Source: CAD feature listing. Evaluate the final solid. Frame: model axes, mm. A direction names the side the tool comes from. Give positions to 0.01 mm unless a question says otherwise; leave off trailing zeros. Order: outer loops, then holes, each group sorted by start corner. A loop starts at its lowest first (then second) coordinate and runs counter-clockwise, first axis right, second up.
```python
from build123d import *

# Parameters (mm, degrees)
EXTRUDE_1_DEPTH = 180


with BuildPart() as part:
    # 草图1 → 凸台-拉伸1 (new body)
    with BuildSketch(Plane.XY):
        Polygon((0, 0), (110, 0), (110, -30), (102, -30), (102, -8), (0, -8), align=None)
    extrude(amount=EXTRUDE_1_DEPTH)


solid = part.part
```
1) Section query A-A, the plane z = 44. Return the cut outline in (x, y).
Report:
outline: (0, -8) - (102, -8) - (102, -30) - (110, -30) - (110, 0) - (0, 0) - close
2) Material intervals for L1, parallel to Y at x = 17.5, z = 57; L2, parallel to X at y = -12.25, z = 154, sorted ascending.
Report:
L1: y = -8 to 0
L2: x = 102 to 110
3) Section query B-B, the plane x = 56. Return the cut outline in (y, z).
Report:
outline: (-8, 0) - (0, 0) - (0, 180) - (-8, 180) - close
4) Pin query (flat end, axial travel): pin 1 (10 mm diameter, centred on x = 44.5, z = 71, fed in from -Y); pin 2 (11 mm diameter, centred on y = -19, z = 55, fed in from -X). Return the tip coordinate at first contact, or that it passes through.
Report:
pin 1: stops at y = -8
pin 2: stops at x = 102
5) Section query C-C, the plane y = -16.25. Return the cut outline in (x, z), and give its area (3 significant figures).
Report:
outline: (102, 0) - (110, 0) - (110, 180) - (102, 180) - close
area: 1,440 mm2
6) Reachability of faces 1 (the flat face through (102, -19, 89)), 2 (the flat face through (0, -4, 89)) from +Z, -Z, +X, -X, +Y, -Y: full face, straight path, thin tool, end or side. Return the list, or none.
Report:
face 1: +Z, -Z, -X, -Y
face 2: +Z, -Z, -X, +Y, -Y
